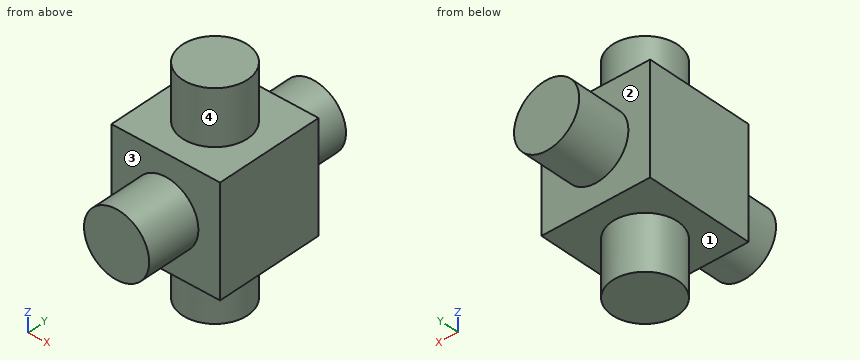
from build123d import *

# Parameters (mm, degrees)
SKETCH_1_W      = 5
SKETCH_1_H      = 5
EXTRUDE_1_DEPTH = 2.5
SKETCH_2_R      = 1.5
EXTRUDE_2_DEPTH = 5
SKETCH_3_R      = 1.5
EXTRUDE_3_DEPTH = 5


with BuildPart() as part:
    # 草图1 → 凸台-拉伸1 (new, symmetric)
    with BuildSketch(Plane.XY):
        Rectangle(SKETCH_1_W, SKETCH_1_H)
    extrude(amount=EXTRUDE_1_DEPTH, both=True)

    # 草图2 → 凸台-拉伸2 (add, symmetric)
    with BuildSketch(Plane(origin=(0, 0, 0), x_dir=(1, 0, 0), z_dir=(0, 1, 0))):
        with Locations(Location((0, 0, 0), (0, 0, 90))):
            Circle(SKETCH_2_R)
    extrude(amount=EXTRUDE_2_DEPTH, both=True)

    # 草图3 → 凸台-拉伸3 (add, symmetric)
    with BuildSketch(Plane.XY):
        Circle(SKETCH_3_R)
    extrude(amount=EXTRUDE_3_DEPTH, both=True)


solid = part.part
Geometry: final body of the model. Coordinates: model frame, mm. Face numbers are marked on the shaded views. A direction names the side the tool comes from. Round coordinates to 2 decimals unless told otherwise and drop trailing zeros. Loops run counter-clockwise (first coordinate to the right, second up) from the corner with the lowest first, then second, coordinate; pieces in that order, holes last. Notation, with made-up numbers: M 58.5,52 L 72.5,52 A29 ccw 72.5,83 Z; hole C 27.25,1 d2. An arc over 180 degrees is marked long. Put each result on its own line as item: value. Start each with the question number.
(1) Contact query for a flat-ended pin moving along its axis: pin 1 Ø1 at (x, y) = (0, 3.5) entering from -Z. Output: stop coordinate, or through.
(2) Section query B-B (x = 0). Return loops of the section in (y, z).
(3) Set-up query: the marked faces 1, 2, 3 and 4. Return all of +Z, -Z, +X, -X, +Y, -Y with unobstructed straight access to the full face (end or side cutting, diameter ignored); none if empty.
(4) Material intervals for line 1 along Y through (x, z) = (0.3, -1.5); line 2 along Y through (x, z) = (0, 3), sorted ascending. Write a range as [from, to].
(5) Section query D-D (y = 2.25). Return loops of the section in (x, z), then the cut area to 3 significant figures.
(6) Section query A-A (y = 0). Return loops of the section in (x, z), then the cut area to 3 significant figures.
Findings below:
1. pin 1: stops at z = -1.5
2. outline: M -5,-1.5 L -2.5,-1.5 L -2.5,-2.5 L -1.5,-2.5 L -1.5,-5 L 1.5,-5 L 1.5,-2.5 L 2.5,-2.5 L 2.5,-1.5 L 5,-1.5 L 5,1.5 L 2.5,1.5 L 2.5,2.5 L 1.5,2.5 L 1.5,5 L -1.5,5 L -1.5,2.5 L -2.5,2.5 L -2.5,1.5 L -5,1.5 Z
3. face 1: -Z
3. face 2: +Y
3. face 3: -Y
3. face 4: +Z
4. line 1: y = [-2.5, 2.5]
4. line 2: y = [-1.5, 1.5]
5. outline: M -2.5,-2.5 L 2.5,-2.5 L 2.5,2.5 L -2.5,2.5 Z
5. area: 25.0 mm2
6. outline: M -2.5,-2.5 L -1.5,-2.5 L -1.5,-5 L 1.5,-5 L 1.5,-2.5 L 2.5,-2.5 L 2.5,2.5 L 1.5,2.5 L 1.5,5 L -1.5,5 L -1.5,2.5 L -2.5,2.5 Z
6. area: 40.0 mm2
